Build history of the part. All positions in model axes, mm. Face numbers are marked on the shaded views. A direction names the side the tool comes from. Give positions to 0.01 mm unless a question says otherwise; leave off trailing zeros. Write each loop counter-clockwise with the first axis right and the second up, starting at its lowest first coordinate (ties: lowest second). Pieces come first, ordered by that corner, then holes. Notation, with made-up numbers: (12, 38.5) -> (32, 38.5) arc R22 cw to (32, 48.5) -> close; hole circle Ø10 at (31, 46). An arc over 180 degrees is marked (long way). One line per question, with ' | ' between items. Start each with the question number.
(1) Drill centre lines: probe 1 along Y at (x, z) = (-38, 69.5); probe 2 along X at (y, z) = (-20, 147). Where is each one in solid material? Low to high. Write a range as from..to.
(2) Band-saw the part on A-A, the plane x = -25. Give the cut face in (y, z).
(3) Band-saw the part on B-B, the plane z = 88.5. Give the cut face in (x, y), and give its area (3 significant figures).
(4) Band-saw the part on D-D, the plane y = -42.5. Give the cut face in (x, z).
(5) Pin check, flat tips, straight feed: P1, Ø8, axis at y = -37.5, z = 78, coming from the +X side; P2, Ø3, axis at x = -6, z = 134, coming from the -Y side. Stop position of each tip, or through.
(6) Tool access for the marked faces 1 and 2: list every direction of +Z, -Z, +X, -X, +Y, -Y with a clear straight run to the whole face (end or side of a thin tool).
(7) Band-saw the part on C-C, the plane x = -16.5. Give the cut face in (y, z).
from build123d import *

# Parameters (mm, degrees)
EXTRUDE_1_DEPTH     = 160
CUT_EXTRUDE_1_DEPTH = 10


with BuildPart() as part:
    # Sketch 1 → Extrude 1 (new body)
    with BuildSketch(Plane.XY):
        Polygon((0, 0), (-50, 0), (-50, -50), (-47, -50), (-47, -3), (0, -3), align=None)
    extrude(amount=EXTRUDE_1_DEPTH)

    # Sketch 2 → Cut-Extrude 1 (cut)
    with BuildSketch(Plane(origin=(0, 0, 0), x_dir=(1, 0, 0), z_dir=(0, 1, 0))):
        with BuildLine():
            ThreePointArc((-28.535533906, -131.464466094), (-28.535533906, -138.535533906), (-21.464466094, -138.535533906))
            Line((-21.464466094, -138.535533906), (-28.535533906, -131.464466094))
        make_face()
        with BuildLine():
            Line((-28.535533906, -131.464466094), (-21.464466094, -138.535533906))
            ThreePointArc((-21.464466094, -138.535533906), (-20.380602337, -136.913417162), (-20, -135))
            ThreePointArc((-20, -135), (-23.086582838, -130.380602337), (-28.535533906, -131.464466094))
        make_face()
    extrude(amount=-CUT_EXTRUDE_1_DEPTH, mode=Mode.SUBTRACT)


solid = part.part
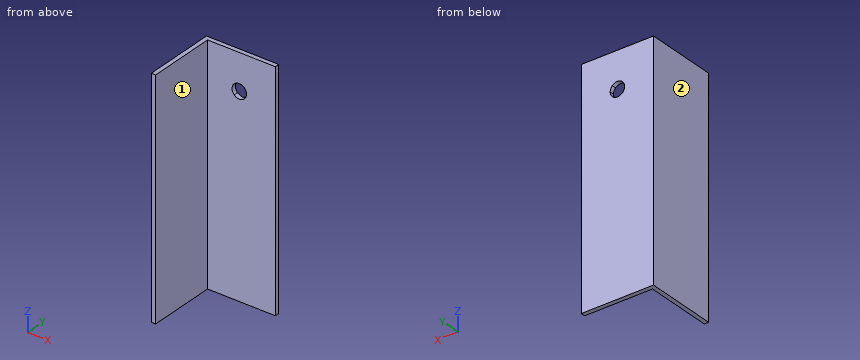
Results:
1) probe 1: y = -3..0 | probe 2: x = -50..-47
2) outline: (-3, 0) -> (0, 0) -> (0, 130) -> (-3, 130) -> close; (-3, 140) -> (0, 140) -> (0, 160) -> (-3, 160) -> close
3) outline: (-50, -50) -> (-47, -50) -> (-47, -3) -> (0, -3) -> (0, 0) -> (-50, 0) -> close | area: 291 mm²
4) outline: (-50, 0) -> (-47, 0) -> (-47, 160) -> (-50, 160) -> close
5) P1: stops at x = -47 | P2: stops at y = -3
6) face 1: +Z, -Z, +X, -Y | face 2: +Z, -Z, -X, +Y, -Y
7) outline: (-3, 0) -> (0, 0) -> (0, 160) -> (-3, 160) -> close
